from build123d import *

# Parameters (mm, degrees)
SKETCH_1_W      = 90
SKETCH_1_H      = 55
SKETCH_1_R      = 1.65
EXTRUDE_1_DEPTH = 0.8


with BuildPart() as part:
    # 草图1 → 凸台-拉伸1 (new, symmetric)
    with BuildSketch(Plane.XY):
        Rectangle(SKETCH_1_W, SKETCH_1_H)
        with Locations((-40, -22.5)):
            Circle(SKETCH_1_R, mode=Mode.SUBTRACT)
        with Locations((-40, 22.5)):
            Circle(SKETCH_1_R, mode=Mode.SUBTRACT)
        with Locations((40, -22.5)):
            Circle(SKETCH_1_R, mode=Mode.SUBTRACT)
        with Locations((40, 22.5)):
            Circle(SKETCH_1_R, mode=Mode.SUBTRACT)
    extrude(amount=EXTRUDE_1_DEPTH, both=True)


solid = part.part
Input: part model. Units: mm. Frame: model coordinates. Coordinates: 2 decimals unless noted, no trailing zeros. Loops run counter-clockwise (first coordinate to the right, second up) from the corner with the lowest first, then second, coordinate; pieces in that order, holes last. Notation, with made-up numbers: (64.25, 65) -> (96.25, 65) arc R26 ccw to (96.25, 90) -> close; hole circle Ø8 at (22, -32.75). An arc over 180 degrees is marked (long way). One line per item, written item: value.
(1) Ray query, line 1 along Y through (x, z) = (40, -0.3). Return the intervals inside material, ascending.
Answer below:
line 1: y = -27.5 to -24.15, -20.85 to 20.85, 24.15 to 27.5
(2) Cut plane A-A (x = 40). Output: boundary loops of the cut face in (y, z), then the cut area to 3 significant figures.
Answer below:
outline: (-27.5, -0.8) -> (-24.15, -0.8) -> (-24.15, 0.8) -> (-27.5, 0.8) -> close; (-20.85, -0.8) -> (20.85, -0.8) -> (20.85, 0.8) -> (-20.85, 0.8) -> close; (24.15, -0.8) -> (27.5, -0.8) -> (27.5, 0.8) -> (24.15, 0.8) -> close
area: 77.4 mm2
(3) Cut plane B-B (y = 22.5). Output: boundary loops of the cut face in (x, z), then the cut area to 3 significant figures.
Answer below:
outline: (-45, -0.8) -> (-41.65, -0.8) -> (-41.65, 0.8) -> (-45, 0.8) -> close; (-38.35, -0.8) -> (38.35, -0.8) -> (38.35, 0.8) -> (-38.35, 0.8) -> close; (41.65, -0.8) -> (45, -0.8) -> (45, 0.8) -> (41.65, 0.8) -> close
area: 133 mm2
(4) Draft query along Y for faces 1 (the face through (-1, 0, -0.8)), 2 (the face through (38.784, 23.615, -0.011)), 3 (the face through (-1, -27.5, 0)). Return one class per face: pulls with the +Y half, pulls with the -Y half, needs draft (parallel to the pull), parting line crosses it, or undercut.
Answer below:
face 1: needs draft
face 2: undercut
face 3: pulls with the -Y half
